CAD build for the part. Positions are in the model's coordinates, mm. A direction names the side the tool comes from. Give positions to 0.01 mm unless a question says otherwise; leave off trailing zeros. Order: outer loops, then holes, each group sorted by start corner. A loop starts at its lowest first (then second) coordinate and runs counter-clockwise, first axis right, second up.
from build123d import *

# Parameters (mm, degrees)
SKETCH1_W           = 140
SKETCH1_H           = 125
BOSS_EXTRUDE1_DEPTH = 8
SKETCH2_R           = 22.5
CUT_EXTRUDE1_DEPTH  = 8
CUT_EXTRUDE2_DEPTH  = 8
LPATTERN1_COUNT     = 2
LPATTERN1_PITCH     = 72
SKETCH4_W           = 48
SKETCH4_H           = 25
CUT_EXTRUDE3_DEPTH  = 8
FILLET1_R           = 10


with BuildPart() as part:
    # Sketch1 → Boss-Extrude1 (new body)
    with BuildSketch(Plane.XY):
        with Locations((70, -62.5)):
            Rectangle(SKETCH1_W, SKETCH1_H)
    extrude(amount=BOSS_EXTRUDE1_DEPTH)

    # Sketch2 → Cut-Extrude1 (cut)
    with BuildSketch(Plane.XY.offset(8)):
        with Locations((66, -66)):
            Circle(SKETCH2_R)
    extrude(amount=-CUT_EXTRUDE1_DEPTH, mode=Mode.SUBTRACT)

    # Sketch3 → Cut-Extrude2 (cut)
    with BuildSketch(Plane.XY.offset(8)):
        with BuildLine():
            Line((35, -96), (35, -116))
            ThreePointArc((35, -116), (30, -121), (25, -116))
            Line((25, -116), (25, -96))
            ThreePointArc((25, -96), (30, -91), (35, -96))
        make_face()
    cut_extrude2 = extrude(amount=-CUT_EXTRUDE2_DEPTH, mode=Mode.SUBTRACT)

    # LPattern1: Cut-Extrude2 ×2
    with Locations(*[(i * LPATTERN1_PITCH, 0, 0) for i in range(1, LPATTERN1_COUNT)]):
        add(cut_extrude2, mode=Mode.SUBTRACT)

    # Sketch4 → Cut-Extrude3 (cut)
    with BuildSketch(Plane.XY.offset(8)):
        with Locations((116, -12.5)):
            Rectangle(SKETCH4_W, SKETCH4_H)
    extrude(amount=-CUT_EXTRUDE3_DEPTH, mode=Mode.SUBTRACT)

    # Fillet1
    fillet1_edges = [part.edges().sort_by_distance(p)[0] for p in [
        (92, -25, 4),
    ]]
    fillet(fillet1_edges, radius=FILLET1_R)


solid = part.part
1. Mould opens along X. For faces 1 (the flat face through (25, -106, 4)), 2 (the flat face through (0, -63, 4)), 3 (the flat face through (45, 0, 4)) say: released by +X, released by -X, zero draft, split by the parting line, or undercut.
2. Saw through at C-C on z = 6.5. Give the cut face in (x, y), plus the area to 3 significant figures.
3. 3-axis set-ups, long thin cutter, end or side, ignore diameter. For faces 4 (the flat face through (121, -25, 4)), 5 (the flat face through (97, -106, 4)), 6 (the flat face through (69, -125, 4)): which of +Z, -Z, +X, -X, +Y, -Y reach the whole face in a straight line?
4. Saw through at D-D on y = -66. Give the cut face in (x, z), plus the area to 3 significant figures.
5. Saw through at A-A on x = 30. Give the cut face in (y, z).
6. Saw through at B-B on y = -100. Give the cut face in (x, z), plus the area to 3 significant figures.
7. Pin check, flat tips, straight feed: P1, Ø1.5, axis at x = 124.5, y = -64, coming from the -Z side; P2, Ø1, axis at x = 120, z = 3.5, coming from the +Y side. Stop position of each tip, or through.
8. Wall check: line 1 (X direction, y = -106, z = 4.25); line 2 (Y direction, x = 66, z = 2.5); line 3 (Y direction, x = 27, z = 6.25). Give the ranges that are in metal, low to high.
Reported:
1. face 1: undercut
1. face 2: released by -X
1. face 3: zero draft
2. outline: (0, -125) - (140, -125) - (140, -25) - (102, -25) arc R10 cw to (92, -15) - (92, 0) - (0, 0) - close; hole (25, -116) arc R5 ccw to (35, -116) - (35, -96) arc R5 ccw to (25, -96) - close; hole circle Ø45 at (66, -66); hole (97, -116) arc R5 ccw to (107, -116) - (107, -96) arc R5 ccw to (97, -96) - close
2. area: 14,200 mm2
3. face 4: +Z, -Z, +X, +Y
3. face 5: +Z, -Z
3. face 6: +Z, -Z, +X, -X, -Y
4. outline: (0, 0) - (43.5, 0) - (43.5, 8) - (0, 8) - close; (88.5, 0) - (140, 0) - (140, 8) - (88.5, 8) - close
4. area: 760 mm2
5. outline: (-125, 0) - (-121, 0) - (-121, 8) - (-125, 8) - close; (-91, 0) - (0, 0) - (0, 8) - (-91, 8) - close
6. outline: (0, 0) - (25, 0) - (25, 8) - (0, 8) - close; (35, 0) - (97, 0) - (97, 8) - (35, 8) - close; (107, 0) - (140, 0) - (140, 8) - (107, 8) - close
6. area: 960 mm2
7. P1: stops at z = 0
7. P2: stops at y = -25
8. line 1: x = 0 to 25, 35 to 97, 107 to 140
8. line 2: y = -125 to -88.5, -43.5 to 0
8. line 3: y = -125 to -120, -92 to 0
